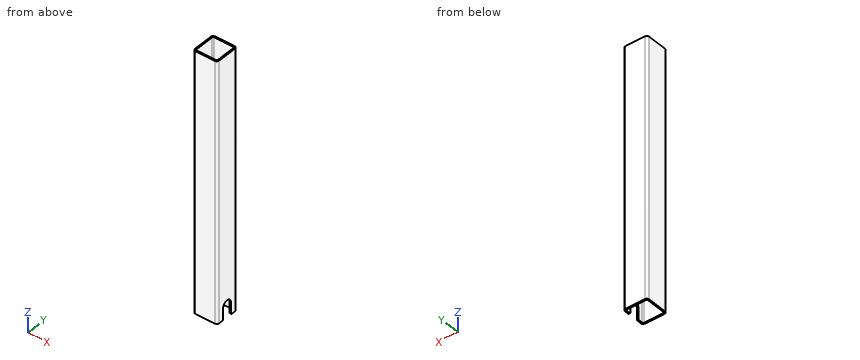
```python
from build123d import *

# Parameters (mm, degrees)
EXTRUDE_1_DEPTH     = 2150
CUT_EXTRUDE_2_DEPTH = 12
FILLET_1_R          = 10


with BuildPart() as part:
    # 草图1 → 凸台-拉伸1 (new body)
    with BuildSketch(Plane.XY):
        with BuildLine():
            Line((-80, 100), (80, 100))
            ThreePointArc((80, 100), (94.142135624, 94.142135624), (100, 80))
            Line((100, 80), (100, -80))
            ThreePointArc((100, -80), (94.142135624, -94.142135624), (80, -100))
            Line((80, -100), (-80, -100))
            ThreePointArc((-80, -100), (-94.142135624, -94.142135624), (-100, -80))
            Line((-100, -80), (-100, 80))
            ThreePointArc((-100, 80), (-94.142135624, 94.142135624), (-80, 100))
        make_face()
        with BuildLine():
            Line((-80, 88), (80, 88))
            ThreePointArc((80, 88), (85.656854249, 85.656854249), (88, 80))
            Line((88, 80), (88, -80))
            ThreePointArc((88, -80), (85.656854249, -85.656854249), (80, -88))
            Line((80, -88), (-80, -88))
            ThreePointArc((-80, -88), (-85.656854249, -85.656854249), (-88, -80))
            Line((-88, -80), (-88, 80))
            ThreePointArc((-88, 80), (-85.656854249, 85.656854249), (-80, 88))
        make_face(mode=Mode.SUBTRACT)
    extrude(amount=EXTRUDE_1_DEPTH)

    # 草图3 → 切除-拉伸2 (cut)
    with BuildSketch(Plane(origin=(100, 0, 0), x_dir=(0, 0, -1), z_dir=(1, 0, 0))):
        with BuildLine():
            Line((-100, 40), (100, 40))
            ThreePointArc((100, 40), (140, 0), (100, -40))
            Line((100, -40), (-100, -40))
            ThreePointArc((-100, -40), (-140, 0), (-100, 40))
        make_face()
    extrude(amount=-CUT_EXTRUDE_2_DEPTH, mode=Mode.SUBTRACT)

    # 圆角1
    fillet_1_edges = [part.edges().sort_by_distance(p)[0] for p in [
        (94, -40, 0),
        (94, 40, 0),
    ]]
    fillet(fillet_1_edges, radius=FILLET_1_R)


solid = part.part
```
Input: part model. Units: mm. Frame: model coordinates. Round coordinates to 2 decimals unless told otherwise and drop trailing zeros. Loops run counter-clockwise (first coordinate to the right, second up) from the corner with the lowest first, then second, coordinate; pieces in that order, holes last.
1) Section query A-A on y = 0. Return the cut outline in (x, z), plus the area to 3 significant figures.
Ans:
outline: (-100, 0) - (-88, 0) - (-88, 2150) - (-100, 2150) - close; (88, 140) - (100, 140) - (100, 2150) - (88, 2150) - close
area: 49,900 mm2
2) Pin query (flat end, axial travel): pin 1 (6 mm diameter, centred on x = 93, z = 55, fed in from -Y); pin 2 (13 mm diameter, centred on x = 91.5, z = 60.5, fed in from +Y). Return the tip coordinate at first contact, or that it passes through.
Ans:
pin 1: stops at y = -97.32
pin 2: stops at y = 99.36
3) Material intervals for line 1 (Y direction, x = 28, z = 1474); line 2 (X direction, y = -85.5, z = 1251.5), sorted ascending.
Ans:
line 1: y = -100 to -88, 88 to 100
line 2: x = -99.23 to -85.81, 85.81 to 99.23
4) Section query B-B on z = 1446.5. Return the cut outline in (x, y).
Ans:
outline: (-100, -80) arc R20 ccw to (-80, -100) - (80, -100) arc R20 ccw to (100, -80) - (100, 80) arc R20 ccw to (80, 100) - (-80, 100) arc R20 ccw to (-100, 80) - close; hole (-88, -80) arc R8 ccw to (-80, -88) - (80, -88) arc R8 ccw to (88, -80) - (88, 80) arc R8 ccw to (80, 88) - (-80, 88) arc R8 ccw to (-88, 80) - close
5) Section query C-C on x = -27.5. Return the cut outline in (y, z), plus the area to 3 significant figures.
Ans:
outline: (-100, 0) - (-88, 0) - (-88, 2150) - (-100, 2150) - close; (88, 0) - (100, 0) - (100, 2150) - (88, 2150) - close
area: 51,600 mm2
